The model under review builds one solid part; all positions refer to its coordinate system, in mm. Round coordinates to 2 decimals unless told otherwise and drop trailing zeros. Order: outer loops, then holes, each group sorted by start corner. A loop starts at its lowest first (then second) coordinate and runs counter-clockwise, first axis right, second up. Notation, with made-up numbers: M 89.5,4 L 135.5,4 A19 cw 135.5,38 Z; hole C -14,24.25 d9. An arc over 180 degrees is marked long. Answer as a JSON object with one key per item and string values. Group by question number.
1. To check wall thickness, follow probe 1 along X at (y, z) = (0.75, 34.75); probe 2 along X at (y, z) = (0.2, 36); probe 3 along X at (y, z) = (0.7, 0). State the ranges of each line that lie inside material, in increasing order. Write a range as [from, to].
2. Add section C-C on z = 0. State the section outline as (x, y) points, and give its area (3 significant figures).
3. Add section A-A on z = 34.75. State the section outline as (x, y) points.
4. Add section B-B on x = 0. State the section outline as (y, z) points, and give its area (3 significant figures).
```python
from build123d import *

# Parameters (mm, degrees)
SKETCH1_W           = 110.5
SKETCH1_H           = 110.5
SKETCH1_R           = 2.55
SKETCH1_R_2         = 1.5
BOSS_EXTRUDE1_DEPTH = 1


with BuildPart() as part:
    # Sketch1 → Boss-Extrude1 (new body)
    with BuildSketch(Plane(origin=(0, 0, 0), x_dir=(1, 0, 0), z_dir=(0, 1, 0))):
        Rectangle(SKETCH1_W, SKETCH1_H)
        with Locations(Location((0, 0, 0), (0, 0, 270))):
            Circle(SKETCH1_R, mode=Mode.SUBTRACT)
        with Locations(Location((-11.5, -34.75, 0), (0, 0, 270))):
            Circle(SKETCH1_R_2, mode=Mode.SUBTRACT)
        with Locations(Location((11.5, -34.75, 0), (0, 0, 270))):
            Circle(SKETCH1_R_2, mode=Mode.SUBTRACT)
    extrude(amount=BOSS_EXTRUDE1_DEPTH)


solid = part.part
```
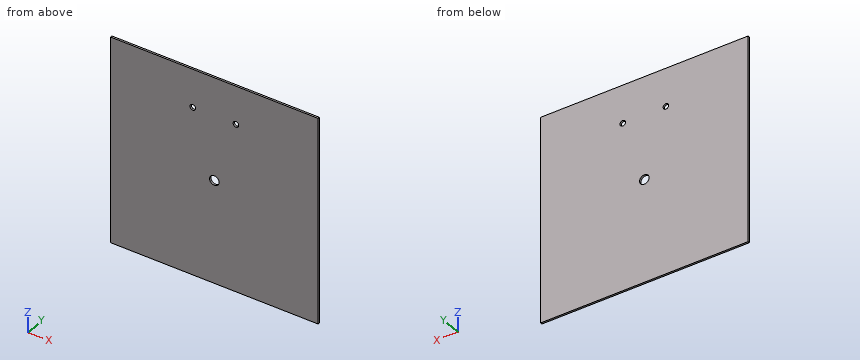
Recorded:
{
 "1": {"probe 1": "x = [-55.25, -13], [-10, 10], [13, 55.25]", "probe 2": "x = [-55.25, -12.33], [-10.67, 10.67], [12.33, 55.25]", "probe 3": "x = [-55.25, -2.55], [2.55, 55.25]"},
 "2": {"outline": "M -55.25,0 L -2.55,0 L -2.55,1 L -55.25,1 Z; M 2.55,0 L 55.25,0 L 55.25,1 L 2.55,1 Z", "area": "105 mm²"},
 "3": {"outline": "M -55.25,0 L -13,0 L -13,1 L -55.25,1 Z; M -10,0 L 10,0 L 10,1 L -10,1 Z; M 13,0 L 55.25,0 L 55.25,1 L 13,1 Z"},
 "4": {"outline": "M 0,-55.25 L 1,-55.25 L 1,-2.55 L 0,-2.55 Z; M 0,2.55 L 1,2.55 L 1,55.25 L 0,55.25 Z", "area": "105 mm²"}
}
